Can you work these out from the drawing? Everything is in mm from the part's minimum corner. Round coordinates to 2 decimals unless told otherwise and drop trailing zeros. Loops run counter-clockwise (first coordinate to the right, second up) from the corner with the lowest first, then second, coordinate; pieces in that order, holes last. Notation, with made-up numbers: (-24, -27.75) - (5, -27.75) arc R26 cw to (5, -5.75) - close; hole circle Ø4 at (50, 14). An arc over 180 degrees is marked (long way). Put each result on its own line as item: value. Start each with the question number.
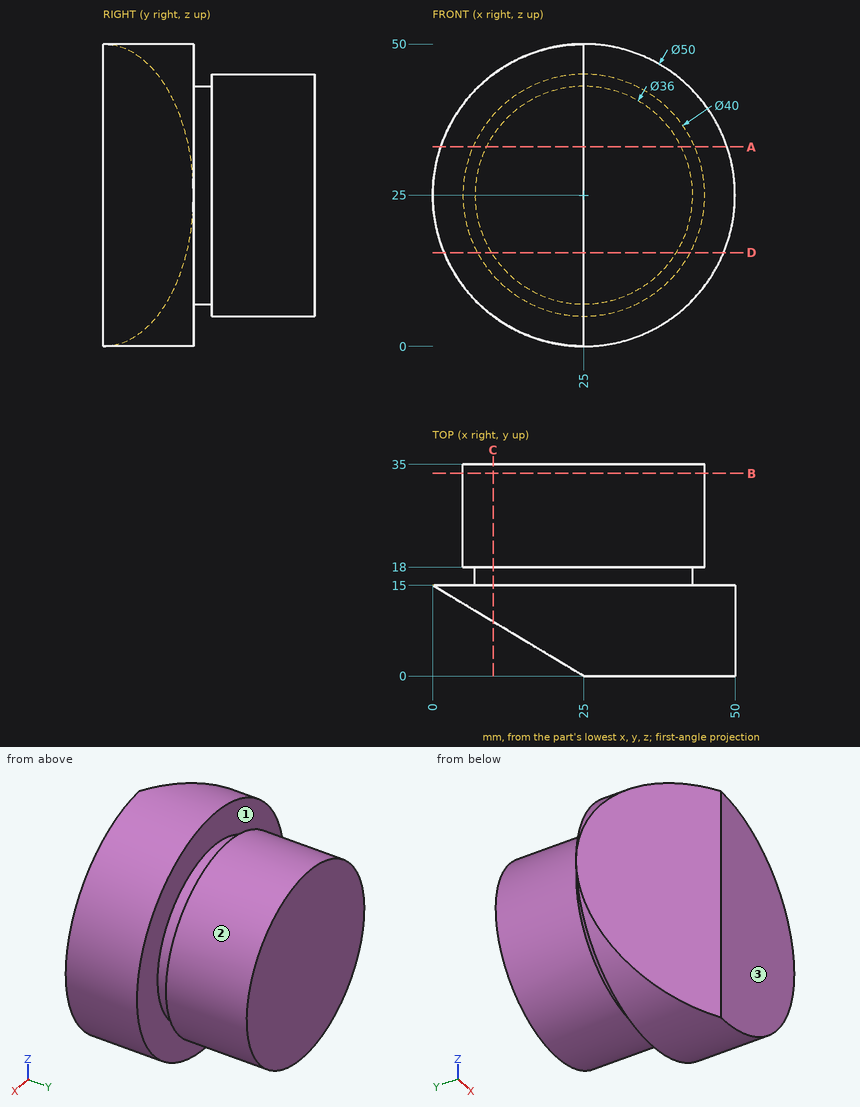
Item 1: I need wall thicknesses on line 1 (Y direction, x = 31.5, z = 7.5); line 2 (Z direction, x = 41, y = 17.5); line 3 (Y direction, x = 29.5, z = 5). Which ranges of each line are inside material? Lowest first, please. Write a range as from..to.
Item 2: Will these pins go through, and if not, where does the flat tip stop? P1, Ø8, axis at x = 43, y = 4, coming from the -Z side; P2, Ø5, axis at x = 12.5, y = 4.5, coming from the -Z side; P3, Ø2, axis at x = 20, z = 27.5, coming from the -Y side; P4, Ø4, axis at x = 34, z = 17.5, coming from the -Y side.
Item 3: Suppose I cut it at A-A, the plane z = 33. List the corners of the cut face in (x, y) for me, then the cut area to 3 significant figures.
Item 4: Suppose I cut it at C-C, the plane x = 10. List the corners of the cut face in (y, z) for me.
Item 5: Suppose I cut it at B-B, the plane y = 33.5. List the corners of the cut face in (x, z) for me, then the cut area to 3 significant figures.
Item 6: Suppose I cut it at D-D, the plane z = 15.5. List the corners of the cut face in (x, y) for me, then the cut area to 3 significant figures.
Item 7: Thinking about a two-plate mould opening in Y: for the marked faces 1, 2 and 3, which applies, released by +Y, released by -Y, zero draft, split by the parting line, or undercut?
Numbers:
1. line 1: 0..15, 18..35
1. line 2: 16.75..33.25
1. line 3: 0..15
2. P1: z = 4.29
2. P2: through
2. P3: y = 2.4
2. P4: y = 0
3. outline: (1.31, 14.21) - (25, 0) - (48.69, 0) - (48.69, 15) - (41.12, 15) - (41.12, 18) - (43.33, 18) - (43.33, 35) - (6.67, 35) - (6.67, 18) - (8.88, 18) - (8.88, 15) - (1.31, 15) - close
3. area: 1,260 mm^2
4. outline: (9, 5) - (15, 5) - (15, 15.05) - (18, 15.05) - (18, 11.77) - (35, 11.77) - (35, 38.23) - (18, 38.23) - (18, 34.95) - (15, 34.95) - (15, 45) - (9, 45) - close
5. outline: circle Ø40 at (25, 25)
5. area: 1,260 mm^2
6. outline: (1.88, 13.87) - (25, 0) - (48.12, 0) - (48.12, 15) - (40.29, 15) - (40.29, 18) - (42.6, 18) - (42.6, 35) - (7.4, 35) - (7.4, 18) - (9.71, 18) - (9.71, 15) - (1.88, 15) - close
6. area: 1,220 mm^2
7. face 1: undercut
7. face 2: zero draft
7. face 3: released by -Y
